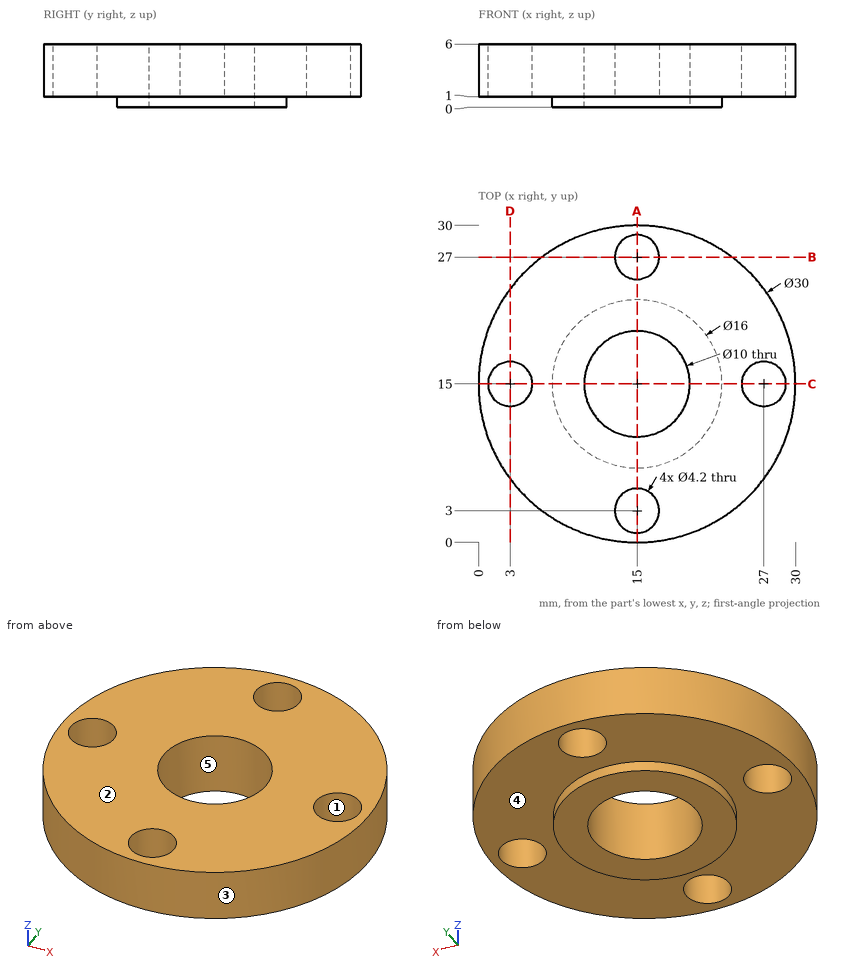
Geometry: see drawing. Coordinates: mm, zero at the bounding-box minimum. A direction names the side the tool comes from. Coordinates: 2 decimals unless noted, no trailing zeros. Loops run counter-clockwise (first coordinate to the right, second up) from the corner with the lowest first, then second, coordinate; pieces in that order, holes last. Notation, with made-up numbers: M -20.5,78 L -6.5,78 A17 ccw -6.5,110 Z; hole C -32.75,53 d8. An arc over 180 degrees is marked long. Answer in a Markdown table with one row per item.
1. Section B-B, the plane y = 27. Output: boundary loops of the cut face in (x, z).
Response:
| item | result |
|---|---|
| outline | M 6,1 L 12.9,1 L 12.9,6 L 6,6 Z; M 17.1,1 L 24,1 L 24,6 L 17.1,6 Z |
2. Draft query along X for the marked faces 1, 2 and 3. Return one class per face: pulls with the +X half, pulls with the -X half, needs draft (parallel to the pull), parting line crosses it, or undercut.
Response:
| item | result |
|---|---|
| face 1 | undercut |
| face 2 | needs draft |
| face 3 | parting line crosses it |
3. Material intervals for line 1 (Y direction, x = 15, z = 3.2); line 2 (X direction, y = 14.5, z = 1.95); line 3 (Y direction, x = 13.75, z = 2.05), sorted ascending.
Response:
| item | result |
|---|---|
| line 1 | y = 0 to 0.9, 5.1 to 10, 20 to 24.9, 29.1 to 30 |
| line 2 | x = 0.01 to 0.96, 5.04 to 10.03, 19.97 to 24.96, 29.04 to 29.99 |
| line 3 | y = 0.05 to 1.31, 4.69 to 10.16, 19.84 to 25.31, 28.69 to 29.95 |
4. Reachability of the marked faces 4 and 5 from +Z, -Z, +X, -X, +Y, -Y: full face, straight path, thin tool, end or side. Return the list, or none.
Response:
| item | result |
|---|---|
| face 4 | -Z |
| face 5 | +Z, -Z |
5. Section A-A, the plane x = 15. Output: boundary loops of the cut face in (y, z).
Response:
| item | result |
|---|---|
| outline | M 0,1 L 0.9,1 L 0.9,6 L 0,6 Z; M 5.1,1 L 7,1 L 7,0 L 10,0 L 10,6 L 5.1,6 Z; M 20,0 L 23,0 L 23,1 L 24.9,1 L 24.9,6 L 20,6 Z; M 29.1,1 L 30,1 L 30,6 L 29.1,6 Z |
6. First-contact query: pin 1 (6.5 mm diameter, centred on x = 3, y = 15, fed in from -Z); pin 2 (2 mm diameter, centred on x = 18, z = 2, fed in from -Y). Flat tips, straight axial feed; report the tip coordinate or a pass-through.
Response:
| item | result |
|---|---|
| pin 1 | stops at z = 1 |
| pin 2 | stops at y = 0.13 |
